Geometry check sheet. Reference: the model listing, model coordinates, mm. A direction names the side the tool comes from. Coordinates: 2 decimals unless noted, no trailing zeros. Loops run counter-clockwise (first coordinate to the right, second up) from the corner with the lowest first, then second, coordinate; pieces in that order, holes last.
from build123d import *

# Parameters (mm, degrees)
SKETCH1_W           = 14
SKETCH1_H           = 35
BOSS_EXTRUDE1_DEPTH = 5.5
SKETCH8_R           = 1.25
SKETCH8_R_2         = 1
CUT_EXTRUDE1_DEPTH  = 1
CUT_EXTRUDE2_DEPTH  = 1.3
SKETCH10_R          = 1.5
SKETCH10_R_2        = 1.25
CUT_EXTRUDE3_DEPTH  = 1
CUT_EXTRUDE4_DEPTH  = 1.5


with BuildPart() as part:
    # Sketch1 → Boss-Extrude1 (new body)
    with BuildSketch(Plane.XY.offset(8)):
        with Locations((2, 0)):
            Rectangle(SKETCH1_W, SKETCH1_H)
    extrude(amount=BOSS_EXTRUDE1_DEPTH)

    # Sketch2 → Revolve1 (revolve)
    with BuildSketch(Plane(origin=(0, 0, 0), x_dir=(0, 0, -1), z_dir=(1, 0, 0)), mode=Mode.PRIVATE) as revolve1_sk:
        Polygon((-13, 8), (-13, 10), (23, 10), (23, 11), (28, 11), (28, 8), align=None)
    revolve(revolve1_sk.sketch.rotate(Axis((0, 8, -28), (0, 0, 1)), 270), axis=Axis((0, 8, -28), (0, 0, 1)))

    # Sketch3 → Revolve2 (revolve)
    with BuildSketch(Plane(origin=(0, 0, 0), x_dir=(0, 0, -1), z_dir=(1, 0, 0)), mode=Mode.PRIVATE) as revolve2_sk:
        Polygon((-13, -8), (-13, -6), (23, -6), (23, -5), (28, -5), (28, -8), align=None)
    revolve(revolve2_sk.sketch.rotate(Axis((0, -8, -28), (0, 0, 1)), 270), axis=Axis((0, -8, -28), (0, 0, 1)))

    # Sketch4 → Cut-Revolve1 (revolve, cut)
    with BuildSketch(Plane(origin=(2, 0, 0), x_dir=(0, 0, -1), z_dir=(1, 0, 0)), mode=Mode.PRIVATE) as cut_revolve1_sk:
        Polygon((-13.5, 14), (-13.5, 15.5), (-13.2295, 15.2295), (-8.2705, 15.2295), (-8, 15.5), (-8, 14), align=None)
    revolve(cut_revolve1_sk.sketch.rotate(Axis((2, 14, 8), (0, 0, 1)), 270), axis=Axis((2, 14, 8), (0, 0, 1)), mode=Mode.SUBTRACT)

    # Sketch5 → Cut-Revolve2 (revolve, cut)
    with BuildSketch(Plane(origin=(2, 0, 0), x_dir=(0, 0, -1), z_dir=(1, 0, 0)), mode=Mode.PRIVATE) as cut_revolve2_sk:
        Polygon((-13.5, -14), (-13.5, -12.5), (-13.2295, -12.7705), (-8.2705, -12.7705), (-8, -12.5), (-8, -14), align=None)
    revolve(cut_revolve2_sk.sketch.rotate(Axis((2, -14, 8), (0, 0, 1)), 270), axis=Axis((2, -14, 8), (0, 0, 1)), mode=Mode.SUBTRACT)

    # Sketch6 → Cut-Revolve3 (revolve, cut)
    with BuildSketch(Plane.XY.offset(10.75), mode=Mode.PRIVATE) as cut_revolve3_sk:
        Polygon((-5, 14), (-5, 15.5), (-4.7295, 15.2295), (8.7295, 15.2295), (9, 15.5), (9, 14), align=None)
    revolve(cut_revolve3_sk.sketch.rotate(Axis((9, 14, 10.75), (-1, 0, 0)), 270), axis=Axis((9, 14, 10.75), (-1, 0, 0)), mode=Mode.SUBTRACT)

    # Sketch7 → Cut-Revolve4 (revolve, cut)
    with BuildSketch(Plane.XY.offset(10.75), mode=Mode.PRIVATE) as cut_revolve4_sk:
        Polygon((-5, -14), (-5, -12.5), (-4.7295, -12.7705), (8.7295, -12.7705), (9, -12.5), (9, -14), align=None)
    revolve(cut_revolve4_sk.sketch.rotate(Axis((9, -14, 10.75), (-1, 0, 0)), 270), axis=Axis((9, -14, 10.75), (-1, 0, 0)), mode=Mode.SUBTRACT)

    # Sketch8 → Cut-Extrude1 (cut)
    with BuildSketch(Plane.XY.offset(13.5)):
        with Locations((0, -8)):
            Circle(SKETCH8_R)
        with Locations((0, -8)):
            Circle(SKETCH8_R_2, mode=Mode.SUBTRACT)
    extrude(amount=-CUT_EXTRUDE1_DEPTH, mode=Mode.SUBTRACT)

    # Sketch9 → Cut-Extrude2 (cut)
    with BuildSketch(Plane.XY.offset(13.5)):
        Polygon((-0.75055535, -8), (-0.375277675, -8.65), (0.375277675, -8.65), (0.75055535, -8), (0.375277675, -7.35), (-0.375277675, -7.35), align=None)
    extrude(amount=-CUT_EXTRUDE2_DEPTH, mode=Mode.SUBTRACT)

    # Sketch10 → Cut-Extrude3 (cut)
    with BuildSketch(Plane(origin=(9, 0, 0), x_dir=(0, 0, -1), z_dir=(1, 0, 0))):
        with Locations((-10.75, 8)):
            Circle(SKETCH10_R)
        with Locations((-10.75, 8)):
            Circle(SKETCH10_R_2, mode=Mode.SUBTRACT)
    extrude(amount=-CUT_EXTRUDE3_DEPTH, mode=Mode.SUBTRACT)

    # Sketch11 → Cut-Extrude4 (cut)
    with BuildSketch(Plane(origin=(9, 0, 0), x_dir=(0, 0, -1), z_dir=(1, 0, 0))):
        Polygon((-11.616025404, 8), (-11.183012702, 7.25), (-10.316987298, 7.25), (-9.883974596, 8), (-10.316987298, 8.75), (-11.183012702, 8.75), align=None)
    extrude(amount=-CUT_EXTRUDE4_DEPTH, mode=Mode.SUBTRACT)


solid = part.part
1) Section check D-D on y = -1.5. Record the cut outline in (x, z), and give its area (3 significant figures).
Data:
outline: (-5, 8) - (9, 8) - (9, 13.5) - (-5, 13.5) - close
area: 77.0 mm2
2) Depth check by flat-ended pin: pin 1 (2 mm diameter, centred on y = -14, z = 10.75, fed in from +X); pin 2 (1.5 mm diameter, centred on x = 2, y = 0.5, fed in from -Z); pin 3 (12 mm diameter, centred on y = 10, z = -9, fed in from -X). Enter the tip coordinate at first touch or a pass-through.
Data:
pin 1: passes through
pin 2: stops at z = 8
pin 3: stops at x = -2
3) Section check B-B on z = -19.5. Record the cut outline in (x, y), and give its area (3 significant figures).
Data:
outline: circle Ø4 at (0, -8); circle Ø4 at (0, 8)
area: 25.1 mm2
4) Access from +Z, -Z, +X, -X, +Y, -Y to the whole of each face (thin tool, end or side, straight path). Record for faces 4 (the cylindrical face through (8.51, 8.05, 12)), 5 (the cylindrical face through (0, -7, 13)), 6 (the cylindrical face through (0, -5, -26)), 7 (the cylindrical face through (-2.07, -13.95, 9.52)), 8 (the cylindrical face through (0, -6, -8)).
Data:
face 4: +X
face 5: +Z
face 6: -Z
face 7: +X, -X
face 8: none
5) Mould release check, pull along Z, two halves, no side actions. Record for faces 1 (the flat face through (9, 7, 11)), 2 (the flat face through (7.5, 8, 11)), 3 (the flat face through (0, -8, 12.2)): +Z half, -Z half, draft (parallel to the pull), parting line (faces both ways), or undercut.
Data:
face 1: draft
face 2: undercut
face 3: +Z half
6) Section check A-A on y = 14. Record the cut outline in (x, z).
Data:
outline: (-5, 8) - (0.5, 8) - (0.77, 8.27) - (0.77, 9.52) - (-4.73, 9.52) - (-5, 9.25) - close; (-5, 12.25) - (-4.73, 11.98) - (0.77, 11.98) - (0.77, 13.23) - (0.5, 13.5) - (-5, 13.5) - close; (3.23, 8.27) - (3.5, 8) - (9, 8) - (9, 9.25) - (8.73, 9.52) - (3.23, 9.52) - close; (3.23, 11.98) - (8.73, 11.98) - (9, 12.25) - (9, 13.5) - (3.5, 13.5) - (3.23, 13.23) - close
7) Material ranges on probe 1 along Y at (x, z) = (8.5, 10.75); probe 2 along Y at (x, z) = (2, 11.85); probe 3 along Z at (x, y) = (-1.25, -14), recorded low to high.
Data:
probe 1: y = -17.5 to -15.23, -12.77 to 6.5, 6.75 to 7.25, 8.75 to 9.25, 9.5 to 12.77, 15.23 to 17.5
probe 2: y = -17.5 to -15.23, -12.77 to 12.77, 15.23 to 17.5
probe 3: z = 8 to 9.52, 11.98 to 13.5
8) Section check C-C on x = 6. Record the cut outline in (y, z), and give its area (3 significant figures).
Data:
outline: (-17.5, 8) - (17.5, 8) - (17.5, 13.5) - (-17.5, 13.5) - close; hole circle Ø2.46 at (-14, 10.75); hole circle Ø2.46 at (14, 10.75)
area: 183 mm2
